from build123d import *

# Parameters (mm, degrees)
SKETCH1_R           = 15
SKETCH1_R_2         = 20
SKETCH1_R_3         = 35
BOSS_EXTRUDE1_DEPTH = 40


with BuildPart() as part:
    # Sketch1 → Boss-Extrude1 (new body)
    with BuildSketch(Plane.XY):
        with BuildLine():
            Line((136298.479378134, -173227.631246443), (136051.215190424, -173587.288246748))
            ThreePointArc((136051.215190424, -173587.288246748), (136040.460393586, -173596.843050045), (136026.493932699, -173600.292382063))
            Line((136026.493932699, -173600.292382063), (135994.358099543, -173600.292382063))
            ThreePointArc((135994.358099543, -173600.292382063), (135980.391638657, -173603.741714079), (135969.636841818, -173613.296517373))
            Line((135969.636841818, -173613.296517373), (135917.386841817, -173689.296517375))
            ThreePointArc((135917.386841817, -173689.296517375), (135915.557431558, -173720.258842949), (135942.10809954, -173736.292382064))
            Line((135942.10809954, -173736.292382064), (136025.44105537, -173736.292382064))
            ThreePointArc((136025.44105537, -173736.292382064), (136028.976589274, -173737.756848164), (136030.44105537, -173741.29238207))
            Line((136030.44105537, -173741.29238207), (136030.44105537, -173760.79238207))
            ThreePointArc((136030.44105537, -173760.79238207), (136031.905521462, -173764.327915975), (136035.441055367, -173765.79238207))
            Line((136035.441055367, -173765.79238207), (136065.44105537, -173765.79238207))
            ThreePointArc((136065.44105537, -173765.79238207), (136068.976589275, -173764.327915968), (136070.441055364, -173760.792382057))
            Line((136070.441055364, -173760.792382057), (136070.441055364, -173709.851867037))
            ThreePointArc((136070.441055364, -173709.851867037), (136071.791118787, -173700.953488864), (136075.71979764, -173692.856002351))
            Line((136075.71979764, -173692.856002351), (136188.781239342, -173528.402996239))
            ThreePointArc((136188.781239342, -173528.402996239), (136199.652035077, -173475.031986515), (136238.252029422, -173436.60440117))
            ThreePointArc((136238.252029422, -173436.60440117), (136257.830557919, -173422.935627875), (136273.610475811, -173405.01501592))
            Line((136273.610475811, -173405.01501592), (136364.402732332, -173272.953551889))
            ThreePointArc((136364.402732332, -173272.953551889), (136354.102207956, -173217.330722066), (136298.479378134, -173227.631246443))
        make_face()
        with Locations((136024.816066991, -173696.292382064)):
            Circle(SKETCH1_R, mode=Mode.SUBTRACT)
        with Locations((135954.816066991, -173696.292382064)):
            Circle(SKETCH1_R, mode=Mode.SUBTRACT)
        with Locations((136100.44105537, -173586.292398967)):
            Circle(SKETCH1_R_2, mode=Mode.SUBTRACT)
        with Locations((136331.44105537, -173250.292398967)):
            Circle(SKETCH1_R_3, mode=Mode.SUBTRACT)
        with BuildLine():
            Line((136121.226562597, -173524.21041858), (136146.693938197, -173482.735767799))
            ThreePointArc((136146.693938197, -173482.735767799), (136169.679901616, -173478.163942115), (136175.848114544, -173500.773879171))
            Line((136175.848114544, -173500.773879171), (136150.47388525, -173542.2345113))
            ThreePointArc((136150.47388525, -173542.2345113), (136126.210129016, -173548.865247662), (136121.226562597, -173524.21041858))
        make_face(mode=Mode.SUBTRACT)
        with BuildLine():
            Line((136223.494638872, -173373.447446962), (136277.473587055, -173294.932613241))
            ThreePointArc((136277.473587055, -173294.932613241), (136302.376683609, -173290.320928694), (136306.988368156, -173315.224025248))
            Line((136306.988368156, -173315.224025248), (136253.009419973, -173393.738858969))
            ThreePointArc((136253.009419973, -173393.738858969), (136228.106323419, -173398.350543516), (136223.494638872, -173373.447446962))
        make_face(mode=Mode.SUBTRACT)
    extrude(amount=BOSS_EXTRUDE1_DEPTH)


solid = part.part
Can you work these out from the model? Positions are in its coordinate system, mm. A direction names the side the tool comes from. Give positions to 0.01 mm unless a question says otherwise; leave off trailing zeros. Loops run counter-clockwise (first coordinate to the right, second up) from the corner with the lowest first, then second, coordinate; pieces in that order, holes last. Notation, with made-up numbers: M -36,-19 L -17,-19 A20 ccw -17,11 Z; hole C -15,14 d7. An arc over 180 degrees is marked long. One line per item, written item: value.
1) Imagine slicing it at A-A on y = -173366.5. Write out the boundary of the cut face in (x, z).
Geometry check:
outline: M 136203.01,0 L 136228.27,0 L 136228.27,40 L 136203.01,40 Z; M 136271.74,0 L 136300.09,0 L 136300.09,40 L 136271.74,40 Z
2) Please list where these lines run through material, in increasing order: line 1 (X direction, y = -173706, z = 20); line 2 (Y direction, x = 135943.5, z = 23.5); line 3 (Y direction, x = 135995.5, z = 19).
Geometry check:
line 1: x = 135912.11 to 135943.38, 135966.25 to 136013.38, 136036.25 to 136070.69
line 2: y = -173736.29 to -173706.14, -173686.45 to -173651.31
line 3: y = -173736.29 to -173600.29
3) Imagine slicing it at D-D on y = -173632.5. Write out the boundary of the cut face in (x, z), and give its area (3 significant figures).
Geometry check:
outline: M 135956.43,0 L 136117.21,0 L 136117.21,40 L 135956.43,40 Z
area: 6,430 mm²
4) I'm going to push flat-ended pins straight in: pin 1 (10 mm diameter, centred on y = -173752, z = 13.5, fed in from -X); pin 2 (1 mm diameter, centred on x = 136218, z = 12.5, fed in from -Y); pin 3 (9.5 mm diameter, centred on x = 136002.5, z = 26.5, fed in from +Y); pin 4 (2 mm diameter, centred on x = 136317, y = -173338, fed in from -Z). Where does each tip first touch, or does it pass through?
Geometry check:
pin 1: stops at x = 136030.44
pin 2: stops at y = -173451.61
pin 3: stops at y = -173600.29
pin 4: stops at z = 0
5) Imagine slicing it at C-C on x = 136018.5. Write out the boundary of the cut face in (y, z), and give its area (3 significant figures).
Geometry check:
outline: M -173736.29,0 L -173709.9,0 L -173709.9,40 L -173736.29,40 Z; M -173682.69,0 L -173600.29,0 L -173600.29,40 L -173682.69,40 Z
area: 4,350 mm²
6) Imagine slicing it at B-B on z = 23. Count the separate pieces of the cut face and the enclosed holes in it, and give its area (3 significant figures).
Geometry check:
separate pieces: 1
enclosed holes: 6
area: 43,800 mm²
7) On a 3-axis mill with a long thin cutter (end or side, diameter ignored), from which of +Z, -Z, +X, -X, +Y, -Y can I reach the whole of each face in a straight line? I mean faces 4 (the face through (136070.441, -173736, 20)), 5 (the face through (135983, -173736.292, 20)), 6 (the face through (136011, -173600.292, 20)), 7 (the face through (136107, -173548, 40)), 8 (the face through (136280.4, -173353.9, 19.7)). Say none if no direction works.
Geometry check:
face 4: +Z, -Z, +X, -Y
face 5: +Z, -Z, -X, -Y
face 6: +Z, -Z, -X, +Y
face 7: +Z, +X, -X, +Y, -Y
face 8: +Z, -Z
8) Thinking about a two-plate mould opening in Y: for faces 1 (the face through (135915.348, -173719.853, 19.72)), 2 (the face through (136126.55, -173549.07, 19.72)), 3 (the face through (136030.441, -173751, 20)), which applies, +Y half, -Y half, draft (parallel to the pull), parting line (faces both ways), or undercut?
Geometry check:
face 1: parting line
face 2: undercut
face 3: draft
